from build123d import *

# Parameters (mm, degrees)
SKETCH_1_W          = 700
SKETCH_1_H          = 760
EXTRUDE_1_DEPTH     = 2
CUT_EXTRUDE_1_DEPTH = 10
SKETCH_3_R          = 15
CUT_EXTRUDE_2_DEPTH = 10


with BuildPart() as part:
    # 草图1 → 凸台-拉伸1 (new body)
    with BuildSketch(Plane.XY):
        Rectangle(SKETCH_1_W, SKETCH_1_H)
    extrude(amount=EXTRUDE_1_DEPTH)

    # 草图2 → 切除-拉伸1 (cut)
    with BuildSketch(Plane.XY.offset(2)):
        with BuildLine():
            Line((-337.75, 375), (-337.75, 365))
            ThreePointArc((-337.75, 365), (-340, 362.75), (-342.25, 365))
            Line((-342.25, 365), (-342.25, 375))
            ThreePointArc((-342.25, 375), (-340, 377.25), (-337.75, 375))
        make_face()
        with BuildLine():
            Line((-342.25, 205), (-342.25, 215))
            ThreePointArc((-342.25, 215), (-340, 217.25), (-337.75, 215))
            Line((-337.75, 215), (-337.75, 205))
            ThreePointArc((-337.75, 205), (-340, 202.75), (-342.25, 205))
        make_face()
        with BuildLine():
            Line((-342.25, 25), (-342.25, 35))
            ThreePointArc((-342.25, 35), (-340, 37.25), (-337.75, 35))
            Line((-337.75, 35), (-337.75, 25))
            ThreePointArc((-337.75, 25), (-340, 22.75), (-342.25, 25))
        make_face()
        with BuildLine():
            Line((337.75, 375), (337.75, 365))
            ThreePointArc((337.75, 365), (340, 362.75), (342.25, 365))
            Line((342.25, 365), (342.25, 375))
            ThreePointArc((342.25, 375), (340, 377.25), (337.75, 375))
        make_face()
        with BuildLine():
            Line((342.25, 205), (342.25, 215))
            ThreePointArc((342.25, 215), (340, 217.25), (337.75, 215))
            Line((337.75, 215), (337.75, 205))
            ThreePointArc((337.75, 205), (340, 202.75), (342.25, 205))
        make_face()
        with BuildLine():
            Line((342.25, 25), (342.25, 35))
            ThreePointArc((342.25, 35), (340, 37.25), (337.75, 35))
            Line((337.75, 35), (337.75, 25))
            ThreePointArc((337.75, 25), (340, 22.75), (342.25, 25))
        make_face()
        with BuildLine():
            Line((-337.75, -315), (-337.75, -305))
            ThreePointArc((-337.75, -305), (-340, -302.75), (-342.25, -305))
            Line((-342.25, -305), (-342.25, -315))
            ThreePointArc((-342.25, -315), (-340, -317.25), (-337.75, -315))
        make_face()
        with BuildLine():
            Line((-337.75, -155), (-337.75, -145))
            ThreePointArc((-337.75, -145), (-340, -142.75), (-342.25, -145))
            Line((-342.25, -145), (-342.25, -155))
            ThreePointArc((-342.25, -155), (-340, -157.25), (-337.75, -155))
        make_face()
        with BuildLine():
            Line((337.75, -315), (337.75, -305))
            ThreePointArc((337.75, -305), (340, -302.75), (342.25, -305))
            Line((342.25, -305), (342.25, -315))
            ThreePointArc((342.25, -315), (340, -317.25), (337.75, -315))
        make_face()
        with BuildLine():
            Line((342.25, -145), (342.25, -155))
            ThreePointArc((342.25, -155), (340, -157.25), (337.75, -155))
            Line((337.75, -155), (337.75, -145))
            ThreePointArc((337.75, -145), (340, -142.75), (342.25, -145))
        make_face()
    extrude(amount=-CUT_EXTRUDE_1_DEPTH, mode=Mode.SUBTRACT)

    # 草图3 → 切除-拉伸2 (cut)
    with BuildSketch(Plane.XY.offset(2)):
        with Locations((0, -280)):
            Circle(SKETCH_3_R)
        with Locations((0, 280)):
            Circle(SKETCH_3_R)
    extrude(amount=-CUT_EXTRUDE_2_DEPTH, mode=Mode.SUBTRACT)


solid = part.part
Input: part model. Units: mm. Frame: model coordinates. Give positions to 0.01 mm unless a question says otherwise; leave off trailing zeros. Loops run counter-clockwise (first coordinate to the right, second up) from the corner with the lowest first, then second, coordinate; pieces in that order, holes last. Notation, with made-up numbers: (-34.5, 78.5) - (-11.5, 78.5) arc R35 ccw to (-11.5, 116.5) - close; hole circle Ø3 at (-23.75, 30). An arc over 180 degrees is marked (long way). Use CSV: the item, a comma, the result in double quotes. Start each with the question number.
Item 1: Section B-B on x = 0. Return loops of the section in (y, z), then the cut area to 3 significant figures.
Item 2: Contact query for a flat-ended pin moving along its axis: P1, Ø2, axis at x = 13, y = 23.5, coming from the -Z side. Output: stop coordinate, or through.
Item 3: Section A-A on y = 280. Return loops of the section in (x, z), then the cut area to 3 significant figures.
Item 4: Mould query, pull axis X, two halves, no side actions, for faces 1 (the cylindrical face through (-1.953, -265.128, 1.014)), 2 (the flat face through (-5, 5, 0)). Classes: pulls with the +X half, pulls with the -X half, needs draft (parallel to the pull), parting line crosses it, or undercut.
Item 5: Line query: line 1 (Y direction, x = 0, z = 1.35); line 2 (Y direction, x = -13, z = 0.7). Output: solid intervals per line, ascending.
Ans:
1,outline,"(-380, 0) - (-295, 0) - (-295, 2) - (-380, 2) - close; (-265, 0) - (265, 0) - (265, 2) - (-265, 2) - close; (295, 0) - (380, 0) - (380, 2) - (295, 2) - close"
1,area,"1,400 mm2"
2,P1,"stops at z = 0"
3,outline,"(-350, 0) - (-15, 0) - (-15, 2) - (-350, 2) - close; (15, 0) - (350, 0) - (350, 2) - (15, 2) - close"
3,area,"1,340 mm2"
4,face 1,"undercut"
4,face 2,"needs draft"
5,line 1,"y = -380 to -295, -265 to 265, 295 to 380"
5,line 2,"y = -380 to -287.48, -272.52 to 272.52, 287.48 to 380"
